```python
from build123d import *

# Parameters (mm, degrees)
SKETCH_1_R          = 10
EXTRUDE_1_DEPTH     = 60
SKETCH_3_R          = 7.5
EXTRUDE_3_DEPTH     = 40
CUT_EXTRUDE_START   = 10
CUT_EXTRUDE_1_DEPTH = 3
CUT_EXTRUDE_START_2 = -10
SKETCH_10_R         = 10
SKETCH_10_R_2       = 7.5
CUT_EXTRUDE_3_DEPTH = 10
CUT_EXTRUDE_START_3 = 7.5
CUT_EXTRUDE_4_DEPTH = 3
EXTRUDE_START       = 20
SKETCH_14_R         = 7.5
EXTRUDE_4_DEPTH     = 20


with BuildPart() as part:
    # 草图1 → 凸台-拉伸1 (new body)
    with BuildSketch(Plane.XY):
        with Locations(Location((0, 0, 0), (0, 0, 180))):
            Circle(SKETCH_1_R)
    extrude(amount=EXTRUDE_1_DEPTH)

    # 草图3 → 凸台-拉伸3 (add)
    with BuildSketch(Plane.XY.offset(60)):
        Circle(SKETCH_3_R)
    extrude(amount=EXTRUDE_3_DEPTH)

    # 草图4 → 切除-拉伸1 (cut)
    with BuildSketch(Plane(origin=(0, 0, 0), x_dir=(0, 0, -1), z_dir=(1, 0, 0)).offset(CUT_EXTRUDE_START)):
        with BuildLine():
            Line((-31, 4), (-19, 4))
            ThreePointArc((-19, 4), (-15, 0), (-19, -4))
            Line((-19, -4), (-31, -4))
            ThreePointArc((-31, -4), (-35, 0), (-31, 4))
        make_face()
    extrude(amount=-CUT_EXTRUDE_1_DEPTH, mode=Mode.SUBTRACT)

    # 草图10 → 切除-拉伸3 (cut)
    with BuildSketch(Plane.XY.offset(60).offset(CUT_EXTRUDE_START_2)):
        Circle(SKETCH_10_R)
        Circle(SKETCH_10_R_2, mode=Mode.SUBTRACT)
    extrude(amount=CUT_EXTRUDE_3_DEPTH, mode=Mode.SUBTRACT)

    # 草图12 → 切除-拉伸4 (cut)
    with BuildSketch(Plane(origin=(0, 0, 0), x_dir=(0, 0, -1), z_dir=(1, 0, 0)).offset(CUT_EXTRUDE_START_3)):
        with BuildLine():
            Line((-84.188029656, 3), (-78.188029656, 3))
            ThreePointArc((-78.188029656, 3), (-75.188029656, 0), (-78.188029656, -3))
            Line((-78.188029656, -3), (-84.188029656, -3))
            ThreePointArc((-84.188029656, -3), (-87.188029656, 0), (-84.188029656, 3))
        make_face()
    extrude(amount=-CUT_EXTRUDE_4_DEPTH, mode=Mode.SUBTRACT)

    # 草图14 → 凸台-拉伸4 (add)
    with BuildSketch(Plane(origin=(0, 0, 0), x_dir=(-1, 0, 0), z_dir=(0, 0, -1)).offset(EXTRUDE_START)):
        with Locations(Location((0, 0, 0), (0, 0, 180))):
            Circle(SKETCH_14_R)
    extrude(amount=-EXTRUDE_4_DEPTH)


solid = part.part
```
Geometry check sheet. Reference: the model listing, model coordinates, mm. A direction names the side the tool comes from. Coordinates: 2 decimals unless noted, no trailing zeros. Write each loop counter-clockwise with the first axis right and the second up, starting at its lowest first coordinate (ties: lowest second). Pieces come first, ordered by that corner, then holes. Notation, with made-up numbers: (-28, -32) -> (-20, -32) arc R13 cw to (-20, -16) -> close; hole circle Ø3 at (-12.5, 38). An arc over 180 degrees is marked (long way). Use CSV: the item, a comma, the result in double quotes. Start each with the question number.
Item 1: Cross-section at A-A, the plane y = 0. Record the cut outline in (x, z).
Item 2: Cross-section at D-D, the plane x = -5.25. Record the cut outline in (y, z), plus the area to 3 significant figures.
Item 3: Cross-section at B-B, the plane x = 0. Record the cut outline in (y, z).
Item 4: Set-up check for faces 1 (the flat face through (8, 4, 25)), 2 (the flat face through (-4, -7, 0)), 3 (the cylindrical face through (-7.493, 0.33, 74.65)): record each of +Z, -Z, +X, -X, +Y, -Y from which the full face is reachable in a straight line by a thin tool's end or side.
Item 5: Mould release check, pull along Z, two halves, no side actions. Record for faces 4 (the cylindrical face through (4.032, -6.324, -10.14)), 5 (the cylindrical face through (6.021, -0.066, 87.187)), 6 (the flat face through (4, 7, 50)): released by +Z, released by -Z, zero draft, split by the parting line, or undercut.
Item 6: Cross-section at C-C, the plane z = 11.5. Record the cut outline in (x, y), plus the area to 3 significant figures.
Item 7: Depth check by flat-ended pin: pin 1 Ø2.5 at (y, z) = (-1, 21) entering from +X; pin 2 Ø6 at (x, z) = (5.5, -6) entering from +Y; pin 3 Ø1.9 at (x, z) = (5.5, 82) entering from -Y. Enter the tip coordinate at first touch or a pass-through.
Item 8: Thickness scan on line 1 (Z direction, x = -6.75, y = 5.25); line 2 (Z direction, x = 4.75, y = 1); line 3 (X direction, y = 5.25, z = 72). Record the ranges inside material, lowest first.
Answers:
1,outline,"(-10, 0) -> (-7.5, 0) -> (-7.5, -20) -> (7.5, -20) -> (7.5, 0) -> (10, 0) -> (10, 15) -> (7, 15) -> (7, 35) -> (10, 35) -> (10, 50) -> (7.5, 50) -> (7.5, 75.19) -> (4.5, 75.19) -> (4.5, 87.19) -> (7.5, 87.19) -> (7.5, 100) -> (-7.5, 100) -> (-7.5, 50) -> (-10, 50) -> close"
2,outline,"(-8.51, 0) -> (-5.36, 0) -> (-5.36, -20) -> (5.36, -20) -> (5.36, 0) -> (8.51, 0) -> (8.51, 50) -> (5.36, 50) -> (5.36, 100) -> (-5.36, 100) -> (-5.36, 50) -> (-8.51, 50) -> close"
2,area,"1,600 mm^2"
3,outline,"(-10, 0) -> (-7.5, 0) -> (-7.5, -20) -> (7.5, -20) -> (7.5, 0) -> (10, 0) -> (10, 50) -> (7.5, 50) -> (7.5, 100) -> (-7.5, 100) -> (-7.5, 50) -> (-10, 50) -> close"
4,face 1,"+X"
4,face 2,"-Z"
4,face 3,"+Z"
5,face 4,"zero draft"
5,face 5,"undercut"
5,face 6,"released by +Z"
6,outline,"circle Ø20 at (0, 0)"
6,area,"314 mm^2"
7,pin 1,"x = 7"
7,pin 2,"y = 7.07"
7,pin 3,"y = -5.96"
8,line 1,"0 to 50"
8,line 2,"-20 to 75.36, 87.02 to 100"
8,line 3,"-5.36 to 5.36"
